from build123d import *

# Parameters (mm, degrees)
CUT_EXTRUDE_1_DEPTH = 4
CUT_EXTRUDE_START   = -1.3
SKETCH_3_R          = 15
SKETCH_3_R_2        = 14.3
CUT_EXTRUDE_2_DEPTH = 1.3
CUT_EXTRUDE_3_DEPTH = 4
SKETCH_5_R          = 15
SKETCH_5_R_2        = 14.3
CUT_EXTRUDE_4_DEPTH = 1.3


with BuildPart() as part:
    # 草图1 → 旋转1 (revolve)
    with BuildSketch(Plane.XY, mode=Mode.PRIVATE) as revolve_1_sk:
        Polygon((0, 0), (0, 15), (110, 15), (110, 17.5), (258, 17.5), (258, 25), (268, 25), (268, 60), (1118, 60), (1118, 25), (1128, 25), (1128, 17.5), (1261, 17.5), (1261, 15), (1293, 15), (1293, 0), align=None)
    revolve(revolve_1_sk.sketch.rotate(Axis((0, 0, 0), (1, 0, 0)), 90), axis=Axis((0, 0, 0), (1, 0, 0)))

    # 草图2 → 切除-拉伸1 (cut)
    with BuildSketch(Plane(origin=(0, 15, 0), x_dir=(1, 0, 0), z_dir=(0, 1, 0))):
        with BuildLine():
            Line((100, 4), (-10, 4))
            Line((-10, 4), (-10, -4))
            Line((-10, -4), (100, -4))
            ThreePointArc((100, -4), (104, 0), (100, 4))
        make_face()
    extrude(amount=-CUT_EXTRUDE_1_DEPTH, mode=Mode.SUBTRACT)

    # 草图3 → 切除-拉伸2 (cut)
    with BuildSketch(Plane.ZY.offset(-12.8).offset(CUT_EXTRUDE_START)):
        Circle(SKETCH_3_R)
        Circle(SKETCH_3_R_2, mode=Mode.SUBTRACT)
    extrude(amount=CUT_EXTRUDE_2_DEPTH, mode=Mode.SUBTRACT)

    # 草图4 → 切除-拉伸3 (cut)
    with BuildSketch(Plane(origin=(0, 15, 0), x_dir=(1, 0, 0), z_dir=(0, 1, 0))):
        with BuildLine():
            Line((1271, 4), (1303, 4))
            Line((1303, 4), (1303, -4))
            Line((1303, -4), (1271, -4))
            ThreePointArc((1271, -4), (1267, 0), (1271, 4))
        make_face()
    extrude(amount=-CUT_EXTRUDE_3_DEPTH, mode=Mode.SUBTRACT)

    # 草图5 → 切除-拉伸4 (cut)
    with BuildSketch(Plane(origin=(1280.2, 0, 0), x_dir=(0, 0, -1), z_dir=(1, 0, 0))):
        with Locations(Location((0, 0, 0), (0, 0, 180))):
            Circle(SKETCH_5_R)
        Circle(SKETCH_5_R_2, mode=Mode.SUBTRACT)
    extrude(amount=-CUT_EXTRUDE_4_DEPTH, mode=Mode.SUBTRACT)


solid = part.part
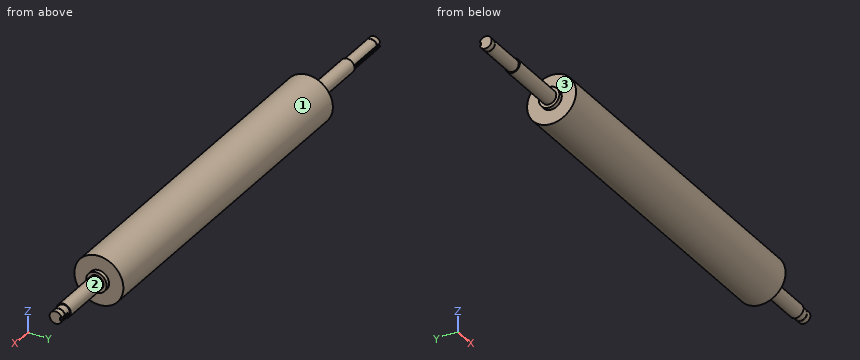
Build history of the part. All positions in model axes, mm. Face numbers are marked on the shaded views. A direction names the side the tool comes from. Round coordinates to 2 decimals unless told otherwise and drop trailing zeros. Loops run counter-clockwise (first coordinate to the right, second up) from the corner with the lowest first, then second, coordinate; pieces in that order, holes last. Notation, with made-up numbers: (29, 17.5) -> (71, 17.5) arc R18 ccw to (71, 34.5) -> close; hole circle Ø9 at (15, 1.5). An arc over 180 degrees is marked (long way). One line per item, written item: value. Start each with the question number.
Q1. Cut at B-B on z = 46. List the corners of the cut face in (x, y).
Q2. Cut at A-A on x = 841.5. List the corners of the cut face in (y, z).
Q3. Probe line 1 along Y through (x, z) = (740, 5); line 2 along X through (y, z) = (-16.5, -39); line 3 along X through (y, z) = (22.5, -1.5). List the from-to ranges inside material, lowest first.
Q4. Drop flat-ended pins along their axis: pin 1 Ø2 at (x, z) = (436, -18) entering from -Y; pin 2 Ø1 at (y, z) = (-15, 37) entering from -X; pin 3 Ø6.5 at (x, z) = (1284, -1.5) entering from +Y; pin 4 Ø14.5 at (y, z) = (-1, 5.5) entering from -X. Give the stop position or say it passes through.
Q5. 3-axis set-ups, long thin cutter, end or side, ignore diameter. For the marked faces 1, 2 and 3: which of +Z, -Z, +X, -X, +Y, -Y reach the whole face in a straight line?
Computed:
1. outline: (268, -38.52) -> (1118, -38.52) -> (1118, 38.52) -> (268, 38.52) -> close
2. outline: circle Ø120 at (0, 0)
3. line 1: -59.79 to 59.79
3. line 2: 268 to 1118
3. line 3: 258 to 1128
4. pin 1: y = -57.54
4. pin 2: x = 268
4. pin 3: y = 14.46
4. pin 4: x = 0
5. face 1: +X, -X
5. face 2: +X
5. face 3: -X
